```python
from build123d import *

# Parameters (mm, degrees)
EXTRUDE_1_DEPTH = 8


with BuildPart() as part:
    # 草图1 → 凸台-拉伸1 (new body)
    with BuildSketch(Plane.XY):
        Polygon((175, -25), (100, -75), (50, -75), (50, -25), (-50, -25), (-50, -75), (-100, -75), (-175, -25), (-175, 60), (-160, 75), (-95, 75), (-80, 60), (-80, 35), (80, 35), (80, 60), (95, 75), (160, 75), (175, 60), align=None)
        with BuildLine():
            Line((-143.8, 43), (-143.8, 33))
            ThreePointArc((-143.8, 33), (-148.3, 28.5), (-152.8, 33))
            Line((-152.8, 33), (-152.8, 43))
            ThreePointArc((-152.8, 43), (-148.3, 47.5), (-143.8, 43))
        make_face(mode=Mode.SUBTRACT)
        with BuildLine():
            Line((-143.8, -7.8), (-143.8, -17.8))
            ThreePointArc((-143.8, -17.8), (-148.3, -22.3), (-152.8, -17.8))
            Line((-152.8, -17.8), (-152.8, -7.8))
            ThreePointArc((-152.8, -7.8), (-148.3, -3.3), (-143.8, -7.8))
        make_face(mode=Mode.SUBTRACT)
        with BuildLine():
            Line((143.8, -7.8), (143.8, -17.8))
            ThreePointArc((143.8, -17.8), (148.3, -22.3), (152.8, -17.8))
            Line((152.8, -17.8), (152.8, -7.8))
            ThreePointArc((152.8, -7.8), (148.3, -3.3), (143.8, -7.8))
        make_face(mode=Mode.SUBTRACT)
        with BuildLine():
            Line((143.8, 43), (143.8, 33))
            ThreePointArc((143.8, 33), (148.3, 28.5), (152.8, 33))
            Line((152.8, 33), (152.8, 43))
            ThreePointArc((152.8, 43), (148.3, 47.5), (143.8, 43))
        make_face(mode=Mode.SUBTRACT)
    extrude(amount=EXTRUDE_1_DEPTH)


solid = part.part
```
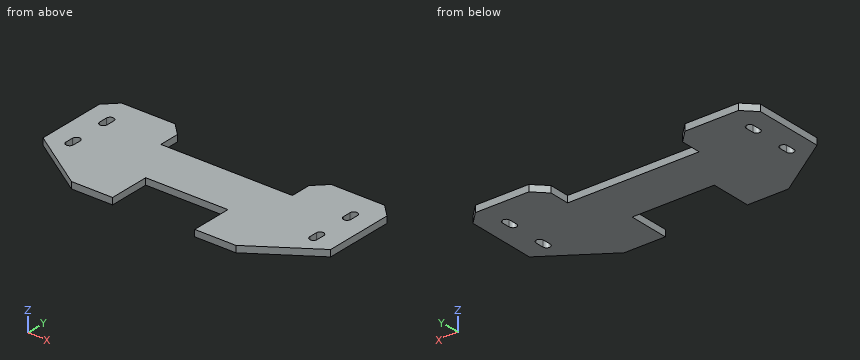
Check sheet for the modelled part. Datum: model origin and axes. Units: mm. Coordinates: 2 decimals unless noted, no trailing zeros. Write each loop counter-clockwise with the first axis right and the second up, starting at its lowest first coordinate (ties: lowest second). Pieces come first, ordered by that corner, then holes. Notation, with made-up numbers: M 89,34 L 100,34 A31 cw 100,59 Z; hole C -31.5,15 d5. An arc over 180 degrees is marked long. Use one line per item in the form item = value.
Item 1: Sectioned sample at B-B, the plane z = 5.75. State how many separate pieces and enclosed holes the cut face has, and give its area (3 significant figures).
Answer below:
separate_pieces = 1
enclosed_holes = 4
area = 36,300 mm^2
Item 2: Material ranges on L1, parallel to X at y = -17, z = 1.5; L2, parallel to X at y = 42, z = 4.75; L3, parallel to X at y = 48, z = 3.75, recorded low to high. Write a range as from..to.
Answer below:
L1 = -175..-152.8, -143.8..143.8, 152.8..175
L2 = -175..-152.8, -143.8..-80, 80..143.8, 152.8..175
L3 = -175..-80, 80..175
Item 3: Sectioned sample at D-D, the plane y = -34. Record the cut outline in (x, z).
Answer below:
outline = M -161.5,0 L -50,0 L -50,8 L -161.5,8 Z; M 50,0 L 161.5,0 L 161.5,8 L 50,8 Z
Item 4: Gauge pin test, flat ends, axial feed: pin 1 Ø1.5 at (x, z) = (19.5, 6.5) entering from -Y; pin 2 Ø4 at (x, z) = (-11, 6) entering from +Y; pin 3 Ø4 at (y, z) = (-56.5, 3) entering from -X; pin 4 Ø10 at (x, y) = (-20, 10.5) entering from -Z. Record the tip position at first contact, or that the pin passes through.
Answer below:
pin_1 = -25
pin_2 = 35
pin_3 = -130.75
pin_4 = 0
Item 5: Sectioned sample at A-A, the plane x = 148.3. Record the cut outline in (y, z), and give its area (3 significant figures).
Answer below:
outline = M -42.8,0 L -22.3,0 L -22.3,8 L -42.8,8 Z; M -3.3,0 L 28.5,0 L 28.5,8 L -3.3,8 Z; M 47.5,0 L 75,0 L 75,8 L 47.5,8 Z
area = 638 mm^2
Item 6: Sectioned sample at C-C, the plane y = -53. Record the cut outline in (x, z), and give its area (3 significant figures).
Answer below:
outline = M -133,0 L -50,0 L -50,8 L -133,8 Z; M 50,0 L 133,0 L 133,8 L 50,8 Z
area = 1,330 mm^2
